The model under review builds one solid part; all positions refer to its coordinate system, in mm. Face numbers are marked on the shaded views. Round coordinates to 2 decimals unless told otherwise and drop trailing zeros. Order: outer loops, then holes, each group sorted by start corner. A loop starts at its lowest first (then second) coordinate and runs counter-clockwise, first axis right, second up.
1) Mouldability with a two-part tool opening along Z and no side actions: class the marked faces 1, 2 and 3 as pulls with the +Z half, pulls with the -Z half, needs draft (parallel to the pull), parting line crosses it, or undercut.
2) To check wall thickness, follow L1, parallel to X at y = 3.25, z = 0; L2, parallel to X at y = 6, z = -1.75; L3, parallel to Z at x = 23.5, y = 8. State the ranges of each line that lie inside material, in increasing order.
3) Consider section B-B (z = 0). Give the boundary of the cut face in (x, y).
4) Consider section C-C (z = -3.5). Give the boundary of the cut face in (x, y), then the cut area to 3 significant figures.
5) Consider section A-A (y = 4). Give the boundary of the cut face in (x, z).
6) Clearance check with a flat-ended pin moving along its axis: P1, Ø1.5, axis at y = 8, z = -1, coming from the +X side. State where the tip first meets the part, or that it passes through.
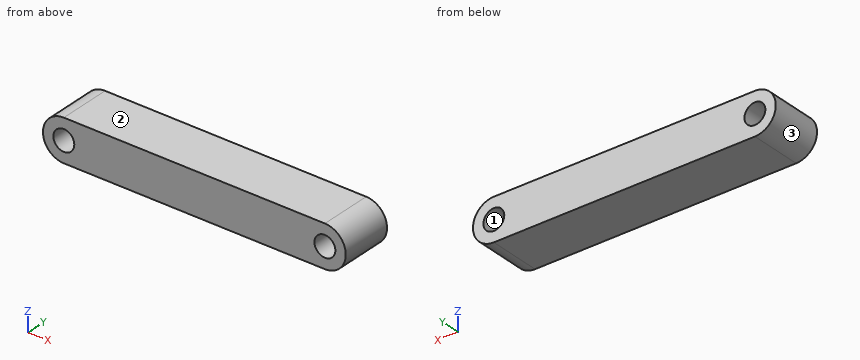
from build123d import *

# Parameters (mm, degrees)
SKETCH1_R           = 2
BOSS_EXTRUDE1_DEPTH = 10


with BuildPart() as part:
    # Sketch1 → Boss-Extrude1 (new body)
    with BuildSketch(Plane(origin=(0, 0, 0), x_dir=(1, 0, 0), z_dir=(0, 1, 0))):
        with BuildLine():
            Line((-25, 4), (25, 4))
            ThreePointArc((25, 4), (29, 0), (25, -4))
            Line((25, -4), (-25, -4))
            ThreePointArc((-25, -4), (-29, 0), (-25, 4))
        make_face()
        with Locations(Location((-25, 0, 0), (0, 0, 270))):
            Circle(SKETCH1_R, mode=Mode.SUBTRACT)
        with Locations(Location((25, 0, 0), (0, 0, 270))):
            Circle(SKETCH1_R, mode=Mode.SUBTRACT)
    extrude(amount=BOSS_EXTRUDE1_DEPTH)


solid = part.part
Answer below:
1. face 1: undercut
1. face 2: pulls with the +Z half
1. face 3: parting line crosses it
2. L1: x = -29 to -27, -23 to 23, 27 to 29
2. L2: x = -28.6 to -25.97, -24.03 to 24.03, 25.97 to 28.6
2. L3: z = -4 to -1.32, 1.32 to 4
3. outline: (-29, 0) - (-27, 0) - (-27, 10) - (-29, 10) - close; (-23, 0) - (23, 0) - (23, 10) - (-23, 10) - close; (27, 0) - (29, 0) - (29, 10) - (27, 10) - close
4. outline: (-26.94, 0) - (26.94, 0) - (26.94, 10) - (-26.94, 10) - close
4. area: 539 mm2
5. outline: (-25, -4) - (25, -4) arc R4 ccw to (25, 4) - (-25, 4) arc R4 ccw to start; hole circle Ø4 at (-25, 0); hole circle Ø4 at (25, 0)
6. P1: stops at x = 28.99
